from build123d import *

# Parameters (mm, degrees)
BRACKET_BODY_DEPTH          = 80
BASE_NOTCH_SKETCH_W         = 15
BASE_NOTCH_SKETCH_H         = 20
BASE_NOTCH_SKETCH_W_2       = 12
BASE_NOTCH_SKETCH_H_2       = 25
BASE_NOTCH_CUT_DEPTH        = 80
SIDE_HOLE_SKETCH_R          = 7.5
SIDE_HOLE_DEPTH             = 40
HALF_LENGTH_BEVEL_CUT_DEPTH = 40


with BuildPart() as part:
    # Bracket Profile Sketch → Bracket Body (new body)
    with BuildSketch(Plane.XY):
        Polygon((0, 0), (50, 0), (50, 5), (10, 50), (0, 50), align=None)
    extrude(amount=BRACKET_BODY_DEPTH)

    # Base Notch Sketch → Base Notch Cut (cut)
    with BuildSketch(Plane.XZ):
        with Locations((42.5, 70)):
            Rectangle(BASE_NOTCH_SKETCH_W, BASE_NOTCH_SKETCH_H)
        with Locations((44, 32.5)):
            Rectangle(BASE_NOTCH_SKETCH_W_2, BASE_NOTCH_SKETCH_H_2)
    extrude(amount=-BASE_NOTCH_CUT_DEPTH, mode=Mode.SUBTRACT)

    # Side Hole Sketch → Side Hole (cut)
    with BuildSketch(Plane.XY.offset(80)):
        with Locations((15, 17)):
            Circle(SIDE_HOLE_SKETCH_R)
    extrude(amount=-SIDE_HOLE_DEPTH, mode=Mode.SUBTRACT)

    # Half-Length Bevel Sketch → Half-Length Bevel Cut (cut)
    with BuildSketch(Plane.ZY):
        Polygon((80, 35), (65, 50), (80, 50), align=None)
    extrude(amount=-HALF_LENGTH_BEVEL_CUT_DEPTH, mode=Mode.SUBTRACT)


solid = part.part
Read the model definition and answer for the solid it produces. Units are mm, in the model's axes. A direction names the side the tool comes from. Coordinates: 2 decimals unless noted, no trailing zeros. Loops run counter-clockwise (first coordinate to the right, second up) from the corner with the lowest first, then second, coordinate; pieces in that order, holes last. Notation, with made-up numbers: (51, 1) -> (85, 1) arc R20 cw to (85, 37) -> close; hole circle Ø10 at (30, -13). An arc over 180 degrees is marked (long way). Answer in a Markdown table with one row per item.
Item 1: For a pull along Z with two mould halves and no side action, classify faces 1 (the flat face through (41, 8, 60)), 2 (the flat face through (43, 7, 45)), 3 (the flat face through (19, 20, 0)), 4 (the flat face through (35, 11, 70)) as released by +Z, released by -Z, zero draft, split by the parting line, or undercut.
Returned:
| item | result |
|---|---|
| face 1 | released by +Z |
| face 2 | undercut |
| face 3 | released by -Z |
| face 4 | zero draft |
Item 2: Straight lines are drawn through the part: line 1 along Z through (x, y) = (41.5, 7.5); line 2 along Z through (x, y) = (35.5, 12); line 3 along X through (y, z) = (11.5, 41). For each, find the intervals that lie inside material, in ascending order. Write a range as [from, to].
Returned:
| item | result |
|---|---|
| line 1 | z = [0, 20], [45, 60] |
| line 2 | z = [0, 60] |
| line 3 | x = [0, 9.9], [20.1, 38] |
Item 3: Each of these flat-tipped pins is pushed along its axis until it touches: P1, Ø1, axis at x = 15, z = 46.5, coming from the +Y side; P2, Ø7.5, axis at x = 15.5, y = 20.5, coming from the +Z side; P3, Ø16, axis at y = 11, z = 66, coming from the +X side. Where does it stop, or does it pass through?
Returned:
| item | result |
|---|---|
| P1 | stops at y = 44.94 |
| P2 | stops at z = 40 |
| P3 | stops at x = 49.37 |
Item 4: A cutting plane is placed at B-B on y = 17. Determine the outline of the cut face in (x, z).
Returned:
| item | result |
|---|---|
| outline | (0, 0) -> (39.33, 0) -> (39.33, 20) -> (38, 20) -> (38, 45) -> (39.33, 45) -> (39.33, 60) -> (35, 60) -> (35, 80) -> (22.5, 80) -> (22.5, 40) -> (7.5, 40) -> (7.5, 80) -> (0, 80) -> close |
Item 5: A cutting plane is placed at D-D on z = 17. Determine the outline of the cut face in (x, y), plus the area to 3 significant figures.
Returned:
| item | result |
|---|---|
| outline | (0, 0) -> (50, 0) -> (50, 5) -> (10, 50) -> (0, 50) -> close |
| area | 1,600 mm^2 |
Item 6: A cutting plane is placed at A-A on z = 58. Determine the outline of the cut face in (x, y).
Returned:
| item | result |
|---|---|
| outline | (0, 0) -> (50, 0) -> (50, 5) -> (10, 50) -> (0, 50) -> close; hole circle Ø15 at (15, 17) |
Item 7: A cutting plane is placed at C-C on x = 15. Determine the outline of the cut face in (y, z) (3 decimals).
Returned:
| item | result |
|---|---|
| outline | (0, 0) -> (44.375, 0) -> (44.375, 70.625) -> (35, 80) -> (24.5, 80) -> (24.5, 40) -> (9.5, 40) -> (9.5, 80) -> (0, 80) -> close |
Item 8: For faces 5 (the flat face through (15, 17, 40)), 6 (the flat face through (38, 9, 32)), 7 (the flat face through (0, 25, 39)), determine the directions among +Z, -Z, +X, -X, +Y, -Y from which every point of the face is accessible in a straight line to the end or side of a thin tool.
Returned:
| item | result |
|---|---|
| face 5 | +Z |
| face 6 | +X, +Y, -Y |
| face 7 | +Z, -Z, -X, +Y, -Y |
